The drawing under review shows one solid part. Ordinate dimensions are in mm from its lowest x, y, z. A direction names the side the tool comes from. Coordinates: 2 decimals unless noted, no trailing zeros. Write each loop counter-clockwise with the first axis right and the second up, starting at its lowest first coordinate (ties: lowest second). Pieces come first, ordered by that corner, then holes.
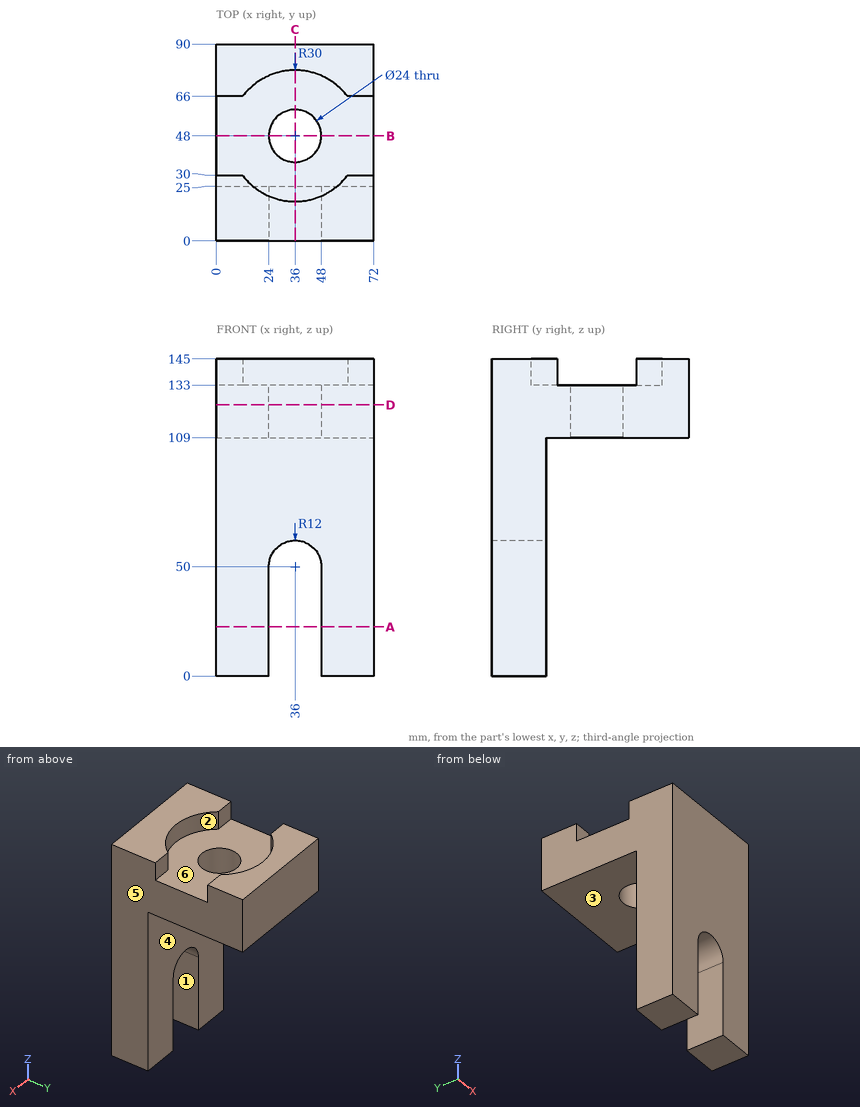
Q1. Clearance check with flat-ended pins moving along their axes: pin 1 Ø8 at (x, y) = (46, 78.5) entering from -Z; pin 2 Ø18 at (x, y) = (22.5, 42) entering from +Z. State where each tip first meets the part, or that it passes through.
Ans:
pin 1: stops at z = 109
pin 2: stops at z = 133
Q2. Tool access review of the marked faces 1, 2 and 3: name each direction out of +Z, -Z, +X, -X, +Y, -Y from which nothing blocks a thin tool from reaching the whole face with its end or side.
Ans:
face 1: -Z, +Y, -Y
face 2: +Z
face 3: -Z, +X, -X, +Y
Q3. Add section D-D (z = 124). State the section outline as (x, y) points.
Ans:
outline: (0, 0) - (72, 0) - (72, 90) - (0, 90) - close; hole circle Ø24 at (36, 48)
Q4. Draft analysis for pull direction X (two halves, no side actions). For the marked faces 4, 5 and 6, state which applies: +X half, -X half, draft (parallel to the pull), parting line (faces both ways), or undercut.
Ans:
face 4: draft
face 5: +X half
face 6: undercut
Q5. Add section A-A (z = 22.5). State the section outline as (x, y) points.
Ans:
outline: (0, 0) - (24, 0) - (24, 25) - (0, 25) - close; (48, 0) - (72, 0) - (72, 25) - (48, 25) - close
Q6. Add section C-C (x = 36). State the section outline as (y, z) points.
Ans:
outline: (0, 62) - (25, 62) - (25, 109) - (36, 109) - (36, 133) - (18, 133) - (18, 145) - (0, 145) - close; (60, 109) - (90, 109) - (90, 145) - (78, 145) - (78, 133) - (60, 133) - close
Q7. Add section B-B (y = 48). State the section outline as (x, z) points.
Ans:
outline: (0, 109) - (24, 109) - (24, 133) - (0, 133) - close; (48, 109) - (72, 109) - (72, 133) - (48, 133) - close
Q8. For probe 1 along X at (y, z) = (15, 25.5); probe 2 along Y at (x, z) = (36, 124.75); probe 3 along Z at (x, y) = (67, 72), list the stretches that pass through material, from the lowest coordinate up.
Ans:
probe 1: x = 0 to 24, 48 to 72
probe 2: y = 0 to 36, 60 to 90
probe 3: z = 109 to 145
